```python
from build123d import *

# Parameters (mm, degrees)
BOSS_EXTRUDE1_DEPTH = 400


with BuildPart() as part:
    # Sketch1 → Boss-Extrude1 (new, symmetric)
    with BuildSketch(Plane(origin=(0, 0, 0), x_dir=(0, 0, -1), z_dir=(1, 0, 0))):
        Polygon((350, 0), (333.923048454, 60), (-50, 60), (-50, 35), (9.378221735, 35), (0, 0), align=None)
    extrude(amount=BOSS_EXTRUDE1_DEPTH, both=True)


solid = part.part
```
Geometry: final body of the model. Coordinates: model frame, mm. Round coordinates to 2 decimals unless told otherwise and drop trailing zeros. Order: outer loops, then holes, each group sorted by start corner. A loop starts at its lowest first (then second) coordinate and runs counter-clockwise, first axis right, second up. Notation, with made-up numbers: (22, 80.5) - (62, 80.5) arc R19 cw to (62, 86.5) - close; hole circle Ø3 at (20.5, 4). An arc over 180 degrees is marked (long way). Write item = value, one per line. Start each with the question number.
Q1. Cut plane A-A on x = -188.5. Return the cut outline in (y, z).
Q2. Pin query (flat end, axial travel): pin 1 (4 mm diameter, centred on x = 276, y = 17.5, fed in from -Z); pin 2 (8 mm diameter, centred on x = -29.5, y = 45, fed in from -Z); pin 3 (3 mm diameter, centred on x = -175.5, z = -240.5, fed in from -Y); pin 4 (1.5 mm diameter, centred on x = -88.5, y = 14.5, fed in from -Z). Return the tip coordinate at first contact, or that it passes through.
Q3. Cut plane B-B on y = 21.5. Return the cut outline in (x, z), and give its area (3 significant figures).
Q4. Ray query, line 1 (Y direction, x = -221, z = 32.5); line 2 (Z direction, x = 268, y = 14); line 3 (Z direction, x = 124.5, y = 43). Return the intervals inside material, ascending. Write a range as from..to.
Q5. Pull-direction query (Y, two-part tool) for faces 1 (the flat face through (-400, 30, -147)), 2 (the flat face through (5.6, 17.745, -4.755)), 3 (the flat face through (6, 0, -173)), 4 (the flat face through (6, 60, -145)); classes: +Y half, -Y half, draft (parallel to the pull), parting line (faces both ways), or undercut.
Outcome:
q1.outline = (0, -350) - (60, -333.92) - (60, 50) - (35, 50) - (35, -9.38) - (0, 0) - close
q2.pin_1 = -345.85
q2.pin_2 = -339.01
q2.pin_3 = 0
q2.pin_4 = -346.32
q3.outline = (-400, -344.24) - (400, -344.24) - (400, -5.76) - (-400, -5.76) - close
q3.area = 271,000 mm^2
q4.line_1 = 35..60
q4.line_2 = -346.25..-3.75
q4.line_3 = -338.48..50
q5.face_1 = draft
q5.face_2 = undercut
q5.face_3 = -Y half
q5.face_4 = +Y half
